from build123d import *

# Parameters (mm, degrees)
SKETCH1_R           = 7.5
BOSS_EXTRUDE1_DEPTH = 15
BOSS_EXTRUDE2_DEPTH = 7
SKETCH3_R           = 7.5
BOSS_EXTRUDE3_DEPTH = 15
SKETCH4_R           = 6.489023352
CUT_EXTRUDE1_DEPTH  = 40.537347476


with BuildPart() as part:
    # Sketch1 → Boss-Extrude1 (new body)
    with BuildSketch(Plane(origin=(0, 0, 0), x_dir=(1, 0, 0), z_dir=(0, 1, 0))):
        with Locations(Location((0, 0, 0), (0, 0, 270))):
            Circle(SKETCH1_R)
    extrude(amount=BOSS_EXTRUDE1_DEPTH)

    # Sketch2 → Boss-Extrude2 (add)
    with BuildSketch(Plane(origin=(0, 15, 0), x_dir=(1, 0, 0), z_dir=(0, 1, 0))):
        Polygon((-9.123012787, 5.267173889), (-9.123012787, -5.267173889), (0, -10.534347777), (9.123012787, -5.267173889), (9.123012787, 5.267173889), (0, 10.534347777), align=None)
    extrude(amount=BOSS_EXTRUDE2_DEPTH)

    # Sketch3 → Boss-Extrude3 (add)
    with BuildSketch(Plane(origin=(0, 22, 0), x_dir=(1, 0, 0), z_dir=(0, 1, 0))):
        with Locations(Location((0, 0, 0), (0, 0, 270))):
            Circle(SKETCH3_R)
    extrude(amount=BOSS_EXTRUDE3_DEPTH)

    # Sketch4 → Cut-Extrude1 (cut, through all)
    with BuildSketch(Plane(origin=(0, 37, 0), x_dir=(1, 0, 0), z_dir=(0, 1, 0))):
        with Locations(Location((0, 0, 0), (0, 0, 270))):
            Circle(SKETCH4_R)
    extrude(amount=-CUT_EXTRUDE1_DEPTH, mode=Mode.SUBTRACT)


solid = part.part
Design review of the part built by this model. Coordinates are the model's own, in mm. A direction names the side the tool comes from. Give positions to 0.01 mm unless a question says otherwise; leave off trailing zeros. Loops run counter-clockwise (first coordinate to the right, second up) from the corner with the lowest first, then second, coordinate; pieces in that order, holes last. Notation, with made-up numbers: (56, -18) - (80, -18) arc R29 ccw to (80, 14) - close; hole circle Ø5 at (-38, -32.5). An arc over 180 degrees is marked (long way). Write item = value, one per line.
1) Tool access review of faces 1 (the face through (0.33, 7.395, -7.493)), 2 (the face through (6, 0, -3)), 3 (the face through (0.33, 29.395, -7.493)): name each direction out of +Z, -Z, +X, -X, +Y, -Y from which nothing blocks a thin tool from reaching the whole face with its end or side.
Result sheet:
face_1 = -Y
face_2 = +Z, -Z, +X, -X, -Y
face_3 = +Y
2) Take a section at A-A on z = 0. State the section outline as (x, y) points, and give its area (3 significant figures).
Result sheet:
outline = (-9.12, 15) - (-7.5, 15) - (-7.5, 0) - (-6.49, 0) - (-6.49, 37) - (-7.5, 37) - (-7.5, 22) - (-9.12, 22) - close; (6.49, 0) - (7.5, 0) - (7.5, 15) - (9.12, 15) - (9.12, 22) - (7.5, 22) - (7.5, 37) - (6.49, 37) - close
area = 97.5 mm2
3) Take a section at C-C on y = 29. State the section outline as (x, z) points.
Result sheet:
outline = circle Ø15 at (0, 0); hole circle Ø12.98 at (0, 0)
4) Clearance check with flat-ended pins moving along their axes: pin 1 Ø1.5 at (y, z) = (33, -6.5) entering from +X; pin 2 Ø6 at (y, z) = (19.5, -7.5) entering from +X; pin 3 Ø8 at (x, y) = (7, 9.5) entering from +Z; pin 4 Ø8 at (x, y) = (-0.5, 4.5) entering from +Z. State where each tip first meets the part, or that it passes through.
Result sheet:
pin_1 = 4.82
pin_2 = 9.12
pin_3 = 6.87
pin_4 = 7.5
5) Draft analysis for pull direction Z (two halves, no side actions). For faces 4 (the face through (-3.95, 18.76, -5.15)), 5 (the face through (4.498, 18.451, 7.938)), 6 (the face through (4.63, 18.45, -7.86)), state which applies: +Z half, -Z half, draft (parallel to the pull), parting line (faces both ways), or undercut.
Result sheet:
face_4 = undercut
face_5 = +Z half
face_6 = -Z half
6) Take a section at B-B on x = -1.75. State the section outline as (y, z) points.
Result sheet:
outline = (0, -7.29) - (15, -7.29) - (15, -9.52) - (22, -9.52) - (22, -7.29) - (37, -7.29) - (37, -6.25) - (0, -6.25) - close; (0, 6.25) - (37, 6.25) - (37, 7.29) - (22, 7.29) - (22, 9.52) - (15, 9.52) - (15, 7.29) - (0, 7.29) - close
7) To check wall thickness, follow line 1 (X direction, y = 27.5, z = 0); line 2 (X direction, y = 17, z = 0); line 3 (Z direction, x = -5, y = 24.5). State the ranges of each line that lie inside material, in increasing order.
Result sheet:
line_1 = -7.5 to -6.49, 6.49 to 7.5
line_2 = -9.12 to -6.49, 6.49 to 9.12
line_3 = -5.59 to -4.14, 4.14 to 5.59
8) Take a section at D-D on z = 8.5. State the section outline as (x, y) points.
Result sheet:
outline = (-3.52, 15) - (3.52, 15) - (3.52, 22) - (-3.52, 22) - close
